```python
from build123d import *

# Parameters (mm, degrees)
BOSS_EXTRUDE1_DEPTH = 10


with BuildPart() as part:
    # Sketch1 → Boss-Extrude1 (new body)
    with BuildSketch(Plane.XY):
        Polygon((0, 0), (20, 0), (90, 125), (90, 145), (20, 145), (0, 125), align=None)
    extrude(amount=BOSS_EXTRUDE1_DEPTH)


solid = part.part
```
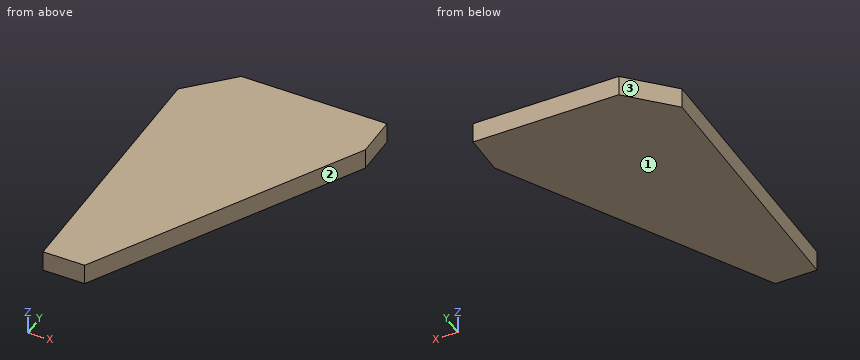
Here's how the part is built. I have some questions about the finished solid (model axes, mm). Face numbers are marked on the shaded views. Coordinates: 2 decimals unless noted, no trailing zeros. Order: outer loops, then holes, each group sorted by start corner. A loop starts at its lowest first (then second) coordinate and runs counter-clockwise, first axis right, second up. Notation, with made-up numbers: M 47.5,70.5 L 102.5,70.5 A7 ccw 102.5,74.5 Z; hole C 28.25,19.5 d10. An arc over 180 degrees is marked long. Answer as a JSON object with one key per item and string values. Group by question number.
(1) For pin 1 (4 mm diameter, centred on y = 52.5, z = 2.5, fed in from +X), with a flat end and sliding along its axis, tell me the tip position at first contact or that it passes through.
(2) If we mould it in two halves opening along X, with no side actions, what happens to the marked faces 1, 2 and 3? For each: released by +X, released by -X, zero draft, split by the parting line, or undercut.
(3) I need wall thicknesses on probe 1 along X at (y, z) = (135, 6.25); probe 2 along X at (y, z) = (112, 3.25); probe 3 along Y at (x, z) = (15, 0.5). Which ranges of each line are inside material? Lowest first, please.
(4) Suppose I cut it at A-A, the plane y = 113.5. Please give me the cut outline in (x, z), then the cut area to 3 significant figures.
(5) Suppose I cut it at B-B, the plane z = 3. Please give me the cut outline in (x, y), then the cut area to 4 significant figures.
(6) Suppose I cut it at C-C, the plane x = 83. Please give me the cut outline in (y, z).
Values found:
{
 "1": {"pin 1": "stops at x = 50.52"},
 "2": {"face 1": "zero draft", "face 2": "released by +X", "face 3": "released by -X"},
 "3": {"probe 1": "x = 10 to 90", "probe 2": "x = 0 to 82.72", "probe 3": "y = 0 to 140"},
 "4": {"outline": "M 0,0 L 83.56,0 L 83.56,10 L 0,10 Z", "area": "836 mm^2"},
 "5": {"outline": "M 0,0 L 20,0 L 90,125 L 90,145 L 20,145 L 0,125 Z", "area": "8,475 mm^2"},
 "6": {"outline": "M 112.5,0 L 145,0 L 145,10 L 112.5,10 Z"}
}
